Can you work these out from the drawing? Everything is in mm from the part's minimum corner. A direction names the side the tool comes from. Round coordinates to 2 decimals unless told otherwise and drop trailing zeros. Write each loop counter-clockwise with the first axis right and the second up, starting at its lowest first coordinate (ties: lowest second). Pieces come first, ordered by that corner, then holes. Notation, with made-up numbers: (87, 5) -> (138, 5) arc R20 ccw to (138, 20) -> close; hole circle Ø7 at (-1.75, -13.75). An arc over 180 degrees is marked (long way). Answer as CSV lines item,"result".
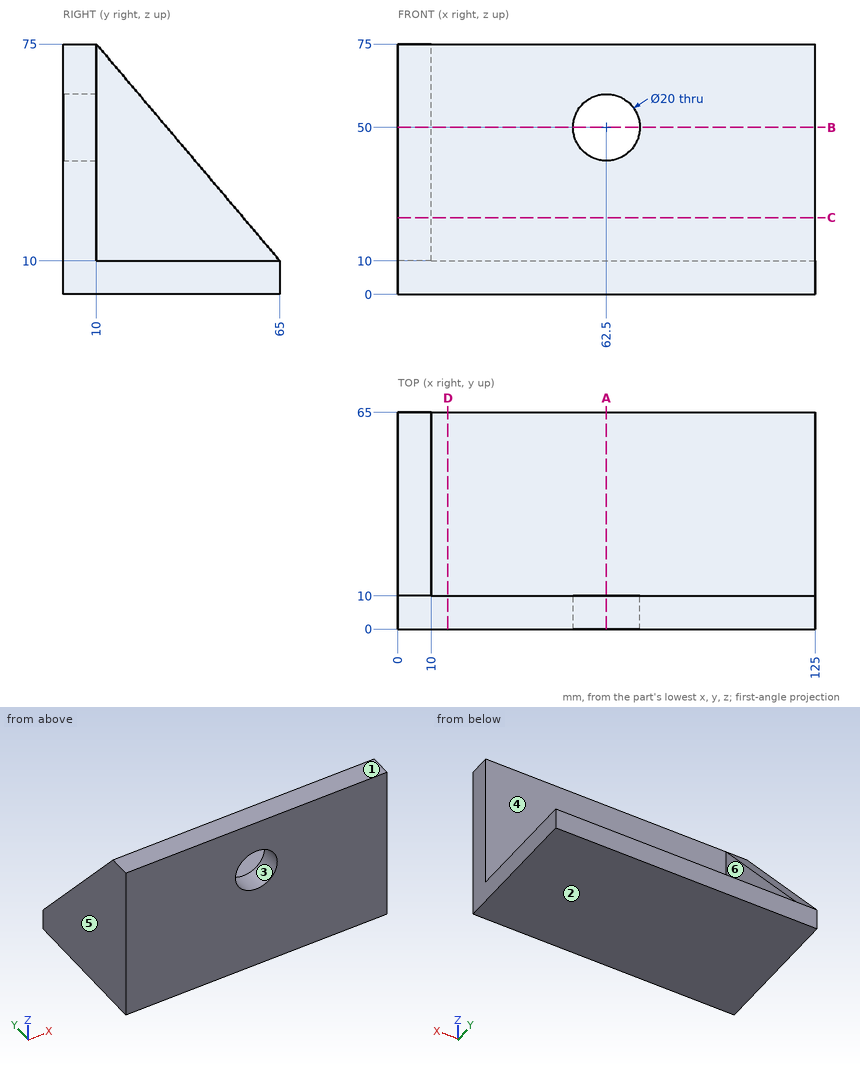
Item 1: Will this pin go through, and if not, where does the flat tip stop? pin 1 (8 mm diameter, centred on x = 51, y = 48, fed in from +Z).
Results found:
pin 1,"stops at z = 10"
Item 2: I need wall thicknesses on L1, parallel to X at y = 5, z = 50; L2, parallel to Z at x = 62, y = 2; L3, parallel to Y at x = 60, z = 19. Which ranges of each line are inside material? Lowest first, please.
Results found:
L1,"x = 0 to 52.5, 72.5 to 125"
L2,"z = 0 to 40.01, 59.99 to 75"
L3,"y = 0 to 10"
Item 3: Suppose I cut it at A-A, the plane x = 62.5. List the corners of the cut face in (y, z) for me, then the cut area to 3 significant figures.
Results found:
outline,"(0, 0) -> (65, 0) -> (65, 10) -> (10, 10) -> (10, 40) -> (0, 40) -> close; (0, 60) -> (10, 60) -> (10, 75) -> (0, 75) -> close"
area,"1,100 mm²"
Item 4: Suppose I cut it at C-C, the plane z = 23. List the corners of the cut face in (x, y) for me.
Results found:
outline,"(0, 0) -> (125, 0) -> (125, 10) -> (10, 10) -> (10, 54) -> (0, 54) -> close"
Item 5: For the marked faces 5 and 6, which set-ups out of +Z, -Z, +X, -X, +Y, -Y let a thin tool reach every point of the face, with its end or its side?
Results found:
face 5,"+Z, -Z, -X, +Y, -Y"
face 6,"+Z, +X, +Y"
Item 6: Suppose I cut it at B-B, the plane z = 50. List the corners of the cut face in (x, y) for me, then the cut area to 3 significant figures.
Results found:
outline,"(0, 0) -> (52.5, 0) -> (52.5, 10) -> (10, 10) -> (10, 31.15) -> (0, 31.15) -> close; (72.5, 0) -> (125, 0) -> (125, 10) -> (72.5, 10) -> close"
area,"1,260 mm²"
Item 7: Suppose I cut it at D-D, the plane x = 15. List the corners of the cut face in (y, z) for me.
Results found:
outline,"(0, 0) -> (65, 0) -> (65, 10) -> (10, 10) -> (10, 75) -> (0, 75) -> close"
Item 8: If we mould it in two halves opening along Z, with no side actions, what happens to the marked faces 1, 2, 3 and 4? For each: pulls with the +Z half, pulls with the -Z half, needs draft (parallel to the pull), parting line crosses it, or undercut.
Results found:
face 1,"pulls with the +Z half"
face 2,"pulls with the -Z half"
face 3,"undercut"
face 4,"needs draft"
